from build123d import *

# Parameters (mm, degrees)
SKETCH2_W               = 366
SKETCH2_H               = 216
SKETCH2_W_2             = 350
SKETCH2_H_2             = 200
BOSS_EXTRUDE1_DEPTH     = 80
SKETCH4_W               = 350
SKETCH4_H               = 200
BOSS_EXTRUDE2_DEPTH     = 2
CUT_EXTRUDE1_DEPTH      = 61
SKETCH6_W               = 120
SKETCH6_H               = 50
CUT_EXTRUDE2_DEPTH      = 61
SKETCH7_R               = 5
SKETCH7_R_2             = 2.5
BOSS_EXTRUDE6_DEPTH     = 11
SKETCH8_R               = 2.5
CUT_EXTRUDE3_DEPTH      = 223.804847344
SKETCH10_R              = 5
BOSS_EXTRUDE7_DEPTH     = 11
SKETCH9_R               = 5
BOSS_EXTRUDE8_DEPTH     = 11
SKETCH11_R              = 2.5
CUT_EXTRUDE4_DEPTH      = 223.804847344
SKETCH12_W              = 2
SKETCH12_H              = 200
EXTRUDE_THIN1_DEPTH     = 66
SKETCH14_W              = 79.91
SKETCH14_H              = 45
BOSS_EXTRUDE9_DEPTH     = 2
LPATTERN1_COUNT         = 3
LPATTERN1_PITCH         = 50
CUT_EXTRUDE5_DEPTH      = 114
CUT_EXTRUDE5_DEPTH_BACK = 26
SKETCH15_R              = 33.472147388
SKETCH16_R              = 20
CUT_EXTRUDE6_DEPTH      = 114
SKETCH20_W              = 113.827039933
SKETCH20_H              = 27.666294428
BOSS_EXTRUDE12_DEPTH    = 41
SKETCH21_R              = 4.720605869
BOSS_EXTRUDE13_DEPTH    = 10


with BuildPart() as part:
    # Sketch2 → Boss-Extrude1 (new body)
    with BuildSketch(Plane(origin=(0, 0, 0), x_dir=(1, 0, 0), z_dir=(0, 1, 0))):
        Rectangle(SKETCH2_W, SKETCH2_H)
        Rectangle(SKETCH2_W_2, SKETCH2_H_2, mode=Mode.SUBTRACT)
    extrude(amount=BOSS_EXTRUDE1_DEPTH)

    # Sketch4 → Boss-Extrude2 (add)
    with BuildSketch(Plane(origin=(0, 80, 0), x_dir=(1, 0, 0), z_dir=(0, 1, 0))):
        Rectangle(SKETCH4_W, SKETCH4_H)
    extrude(amount=-BOSS_EXTRUDE2_DEPTH)

    # Sketch5 → Cut-Extrude1 (cut, symmetric)
    with BuildSketch(Plane.XY.offset(108)):
        with BuildLine():
            Line((58.33950225, 58.901074255), (78.33950225, 58.901074255))
            ThreePointArc((78.33950225, 58.901074255), (83.33950225, 53.901074255), (78.33950225, 48.901074255))
            Line((78.33950225, 48.901074255), (58.33950225, 48.901074255))
            ThreePointArc((58.33950225, 48.901074255), (53.33950225, 53.901074255), (58.33950225, 58.901074255))
        make_face()
    extrude(amount=CUT_EXTRUDE1_DEPTH, both=True, mode=Mode.SUBTRACT)

    # Sketch6 → Cut-Extrude2 (cut, symmetric)
    with BuildSketch(Plane.XY.offset(-100)):
        with Locations((-0.151988162, 42.065744544)):
            Rectangle(SKETCH6_W, SKETCH6_H)
    extrude(amount=CUT_EXTRUDE2_DEPTH, both=True, mode=Mode.SUBTRACT)

    # Sketch7 → Boss-Extrude6 (add)
    # profile 1 of 2: a face of its own
    with BuildSketch(Plane.XZ.offset(-78)):
        with Locations(Location((115, -94.8, 0), (0, 0, 90))):
            Circle(SKETCH7_R)
        with Locations(Location((115, -94.8, 0), (0, 0, 270))):
            Circle(SKETCH7_R_2, mode=Mode.SUBTRACT)
    # profile 2 of 2: a face of its own
    with BuildSketch(Plane.XZ.offset(-78)):
        with Locations(Location((15, -94.8, 0), (0, 0, 90))):
            Circle(SKETCH7_R)
        with Locations(Location((15, -94.8, 0), (0, 0, 270))):
            Circle(SKETCH7_R_2, mode=Mode.SUBTRACT)
    extrude(amount=BOSS_EXTRUDE6_DEPTH)

    # Sketch8 → Cut-Extrude3 (cut, through all)
    with BuildSketch(Plane.XZ.offset(-67)):
        with Locations(Location((15, -94.8, 0), (0, 0, 270))):
            Circle(SKETCH8_R)
        with Locations(Location((115, -94.8, 0), (0, 0, 270))):
            Circle(SKETCH8_R)
    extrude(amount=-CUT_EXTRUDE3_DEPTH, mode=Mode.SUBTRACT)

    # Sketch10 → Boss-Extrude7 (add)
    with BuildSketch(Plane.XZ.offset(-78)):
        with Locations(Location((163.162408198, 93.199516901, 0), (0, 0, 90))):
            Circle(SKETCH10_R)
    extrude(amount=BOSS_EXTRUDE7_DEPTH)

    # Sketch9 → Boss-Extrude8 (add)
    with BuildSketch(Plane.XZ.offset(-78)):
        with Locations(Location((21.965532886, 83.705206519, 0), (0, 0, 90))):
            Circle(SKETCH9_R)
    extrude(amount=BOSS_EXTRUDE8_DEPTH)

    # Sketch11 → Cut-Extrude4 (cut, through all)
    with BuildSketch(Plane.XZ.offset(-67)):
        with Locations(Location((21.965532886, 83.705206519, 0), (0, 0, 270))):
            Circle(SKETCH11_R)
        with Locations(Location((163.162408198, 93.199516901, 0), (0, 0, 270))):
            Circle(SKETCH11_R)
    extrude(amount=-CUT_EXTRUDE4_DEPTH, mode=Mode.SUBTRACT)

    # Sketch12 → Extrude-Thin1 (add)
    with BuildSketch(Plane.XZ.offset(-78)):
        with Locations((-94.091079546, 0)):
            Rectangle(SKETCH12_W, SKETCH12_H)
    extrude(amount=EXTRUDE_THIN1_DEPTH)

    # Sketch14 → Boss-Extrude9 (add, symmetric)
    with BuildSketch(Plane.XY.offset(40)):
        with Locations((-134.390971406, 55.5)):
            Rectangle(SKETCH14_W, SKETCH14_H)
    boss_extrude9 = extrude(amount=BOSS_EXTRUDE9_DEPTH, both=True)

    # LPattern1: Boss-Extrude9 ×3
    with Locations(*[(0, 0, -i * LPATTERN1_PITCH) for i in range(1, LPATTERN1_COUNT)]):
        add(boss_extrude9)

    # Sketch15 → Cut-Extrude5 (cut, two sides: drawn at the far end of the back side and taken through both)
    with BuildSketch(Plane(origin=(0, 0, 38), x_dir=(-1, 0, 0), z_dir=(0, 0, -1)).offset(-CUT_EXTRUDE5_DEPTH_BACK)):
        with Locations((134.390971406, 39.071496759)):
            Circle(SKETCH15_R)
    extrude(amount=CUT_EXTRUDE5_DEPTH + CUT_EXTRUDE5_DEPTH_BACK, mode=Mode.SUBTRACT)

    # Sketch16 → Cut-Extrude6 (cut)
    with BuildSketch(Plane.XY.offset(108)):
        with Locations((-31.393490916, 50.490695355)):
            Circle(SKETCH16_R)
    extrude(amount=-CUT_EXTRUDE6_DEPTH, mode=Mode.SUBTRACT)

    # Sketch20 → Boss-Extrude12 (add)
    with BuildSketch(Plane.XZ.offset(-78)):
        with Locations((7.170460987, -56.94888764)):
            Rectangle(SKETCH20_W, SKETCH20_H)
    extrude(amount=BOSS_EXTRUDE12_DEPTH)

    # Sketch21 → Boss-Extrude13 (add)
    with BuildSketch(Plane(origin=(0, 0, -70.782034854), x_dir=(-1, 0, 0), z_dir=(0, 0, -1))):
        with Locations(Location((-47.399149027, 53.301801825, 0), (0, 0, 180))):
            Circle(SKETCH21_R)
        with Locations(Location((-23.290302455, 53.301801825, 0), (0, 0, 180))):
            Circle(SKETCH21_R)
        with Locations(Location((5.245340735, 53.301801825, 0), (0, 0, 180))):
            Circle(SKETCH21_R)
        with Locations(Location((26.829705026, 53.301801825, 0), (0, 0, 180))):
            Circle(SKETCH21_R)
    extrude(amount=BOSS_EXTRUDE13_DEPTH)


solid = part.part
Model file for the job. Use its own axes, mm. A direction names the side the tool comes from. Round coordinates to 2 decimals unless told otherwise and drop trailing zeros. Order: outer loops, then holes, each group sorted by start corner. A loop starts at its lowest first (then second) coordinate and runs counter-clockwise, first axis right, second up.
(1) Drill centre lines: line 1 (X direction, y = 54, z = -88.5); line 2 (X direction, y = 41, z = -8.5); line 3 (Z direction, x = -162, y = 70.5). Where is each one in solid material? Low to high.
(2) Band-saw the part on B-B (x = -89.5). List the corners of the cut face in (y, z).
(3) 3-axis set-ups, long thin cutter, end or side, ignore diameter. For faces 4 (the face through (-135, 76, -12)), 5 (the face through (59.848, 42, -104)), 6 (the face through (-27, 53, -80.782)), 7 (the face through (68, 58.901, 104)): which of +Z, -Z, +X, -X, +Y, -Y reach the whole face in a straight line?
(4) Band-saw the part on A-A (z = 2.5). List the corners of the cut face in (x, y), then the cut area to 3 significant figures.
(5) Pin check, flat tips, straight feed: pin 1 (4 mm diameter, centred on x = -117.5, z = -73, fed in from -Y); pin 2 (3 mm diameter, centred on x = -6, y = 52.5, fed in from -Z); pin 3 (11 mm diameter, centred on x = 114.5, z = -93.5, fed in from -Y). Stop position of each tip, or through.
(6) Pull direction X, two halves, no side cores. Call faces 1 (the face through (-183, 39, 2)), 2 (the face through (-3, 80, -2)), 3 (the face through (-135.212, 72.534, -9.972)): released by +X, released by -X, zero draft, split by the parting line, or undercut.
Verdict:
1. line 1: x = -183 to -175, -95.09 to -93.09, 175 to 183
1. line 2: x = -183 to -175, -174.35 to -167.81, -100.97 to -93.09, 175 to 183
1. line 3: z = -108 to -100, -62 to -58, -12 to -8, 38 to 42, 100 to 108
2. outline: (0, -108) - (80, -108) - (80, 108) - (0, 108) - (0, 100) - (78, 100) - (78, -100) - (0, -100) - close
3. face 4: -Y
3. face 5: -Z
3. face 6: -Z, -Y
3. face 7: +Z
4. outline: (-183, 0) - (-175, 0) - (-175, 78) - (-95.09, 78) - (-95.09, 12) - (-93.09, 12) - (-93.09, 78) - (175, 78) - (175, 0) - (183, 0) - (183, 80) - (-183, 80) - close
4. area: 2,110 mm2
5. pin 1: stops at y = 78
5. pin 2: stops at z = -80.78
5. pin 3: stops at y = 67
6. face 1: released by -X
6. face 2: zero draft
6. face 3: undercut
